```python
from build123d import *

# Parameters (mm, degrees)
SKETCH1_W           = 85
SKETCH1_H           = 45
BOSS_EXTRUDE1_DEPTH = 2
SKETCH2_W           = 52
SKETCH2_H           = 12
SKETCH2_H_2         = 4.5
SKETCH2_H_3         = 2.5
SKETCH2_H_4         = 13.8
CUT_EXTRUDE1_DEPTH  = 10
SKETCH3_W           = 85
SKETCH3_H           = 13.8
CUT_EXTRUDE2_DEPTH  = 10
SKETCH5_W           = 85
SKETCH5_H           = 5.5
CUT_EXTRUDE4_DEPTH  = 0.1
CHAMFER2_SIZE       = 0.5
CHAMFER2_SIZE2      = 2
CHAMFER3_SIZE       = 2
CHAMFER3_SIZE2      = 0.5
SKETCH8_W           = 85
SKETCH8_H           = 13.8
BOSS_EXTRUDE2_DEPTH = 2
CHAMFER4_SIZE       = 3
SKETCH6_R           = 2
CUT_EXTRUDE5_DEPTH  = 10
CUT_EXTRUDE6_DEPTH  = 6
SKETCH9_R           = 3.25
CUT_EXTRUDE8_DEPTH  = 10
SKETCH4_R           = 2.25
CUT_EXTRUDE3_DEPTH  = 10
SKETCH10_W          = 85
SKETCH10_H          = 8
CUT_EXTRUDE9_DEPTH  = 10
CHAMFER5_SIZE       = 1
CHAMFER5_SIZE2      = 5
CHAMFER6_SIZE       = 2


with BuildPart() as part:
    # Sketch1 → Boss-Extrude1 (new body)
    with BuildSketch(Plane(origin=(0, 0, 0), x_dir=(1, 0, 0), z_dir=(0, 1, 0))):
        Rectangle(SKETCH1_W, SKETCH1_H)
    extrude(amount=BOSS_EXTRUDE1_DEPTH)

    # Sketch2 → Cut-Extrude1 (cut)
    with BuildSketch(Plane(origin=(0, 2, 0), x_dir=(1, 0, 0), z_dir=(0, 1, 0))):
        with Locations((0, -16.5)):
            Rectangle(SKETCH2_W, SKETCH2_H)
        with Locations((0, -4.25)):
            Rectangle(SKETCH2_W, SKETCH2_H_2)
        with Locations((0, 1.75)):
            Rectangle(SKETCH2_W, SKETCH2_H_3)
        with Locations((0, 15.6)):
            Rectangle(SKETCH2_W, SKETCH2_H_4)
    extrude(amount=-CUT_EXTRUDE1_DEPTH, mode=Mode.SUBTRACT)

    # Sketch3 → Cut-Extrude2 (cut)
    with BuildSketch(Plane(origin=(0, 2, 0), x_dir=(1, 0, 0), z_dir=(0, 1, 0))):
        with Locations((0, 15.6)):
            Rectangle(SKETCH3_W, SKETCH3_H)
    extrude(amount=-CUT_EXTRUDE2_DEPTH, mode=Mode.SUBTRACT)

    # Sketch5 → Cut-Extrude4 (cut)
    with BuildSketch(Plane.XZ):
        with Locations((0, 0.75)):
            Rectangle(SKETCH5_W, SKETCH5_H)
    extrude(amount=-CUT_EXTRUDE4_DEPTH, mode=Mode.SUBTRACT)

    # Chamfer2
    chamfer2_edges = [part.edges().sort_by_distance(p)[0] for p in [
        (42.5, 0.05, 3.5),
    ]]
    chamfer2_side = [part.faces().sort_by_distance(p)[0] for p in [
        (42.5, 1.008447858, 6.954688763),
    ]]
    chamfer(chamfer2_edges, length=CHAMFER2_SIZE, length2=CHAMFER2_SIZE2, reference=chamfer2_side[0])

    # Chamfer3
    chamfer3_edges = [part.edges().sort_by_distance(p)[0] for p in [
        (42.5, 0.05, -2),
    ]]
    chamfer3_side = [part.faces().sort_by_distance(p)[0] for p in [
        (34.25, 0.05, -2),
    ]]
    chamfer(chamfer3_edges, length=CHAMFER3_SIZE, length2=CHAMFER3_SIZE2, reference=chamfer3_side[0])

    # Sketch8 → Boss-Extrude2 (add)
    with BuildSketch(Plane(origin=(0, 2, 0), x_dir=(1, 0, 0), z_dir=(0, 1, 0))):
        with Locations((0, 15.6)):
            Rectangle(SKETCH8_W, SKETCH8_H)
    extrude(amount=-BOSS_EXTRUDE2_DEPTH)

    # Chamfer4
    chamfer4_edges = [part.edges().sort_by_distance(p)[0] for p in [
        (-42.5, 1, -22.5),
        (42.5, 1, -22.5),
    ]]
    chamfer(chamfer4_edges, length=CHAMFER4_SIZE)

    # Sketch6 → Cut-Extrude5 (cut)
    with BuildSketch(Plane(origin=(0, 2, 0), x_dir=(1, 0, 0), z_dir=(0, 1, 0))):
        with Locations(Location((-31, 17.5, 0), (0, 0, 270))):
            Circle(SKETCH6_R)
        with Locations(Location((31, 17.5, 0), (0, 0, 270))):
            Circle(SKETCH6_R)
    extrude(amount=-CUT_EXTRUDE5_DEPTH, mode=Mode.SUBTRACT)

    # Sketch7 → Cut-Extrude6 (cut)
    with BuildSketch(Plane(origin=(0, 2, 0), x_dir=(1, 0, 0), z_dir=(0, 1, 0))):
        with BuildLine():
            Line((32, 15.5), (30, 15.5))
            ThreePointArc((30, 15.5), (28, 17.5), (30, 19.5))
            Line((30, 19.5), (32, 19.5))
            ThreePointArc((32, 19.5), (34, 17.5), (32, 15.5))
        make_face()
        with BuildLine():
            Line((-32, 15.5), (-30, 15.5))
            ThreePointArc((-30, 15.5), (-28, 17.5), (-30, 19.5))
            Line((-30, 19.5), (-32, 19.5))
            ThreePointArc((-32, 19.5), (-34, 17.5), (-32, 15.5))
        make_face()
    extrude(amount=-CUT_EXTRUDE6_DEPTH, mode=Mode.SUBTRACT)

    # Sketch9 → Cut-Extrude8 (cut)
    with BuildSketch(Plane(origin=(0, 2, 0), x_dir=(1, 0, 0), z_dir=(0, 1, 0))):
        with Locations(Location((-19, 17, 0), (0, 0, 270))):
            Circle(SKETCH9_R)
        with Locations(Location((19, 17, 0), (0, 0, 270))):
            Circle(SKETCH9_R)
    extrude(amount=-CUT_EXTRUDE8_DEPTH, mode=Mode.SUBTRACT)

    # Sketch4 → Cut-Extrude3 (cut)
    with BuildSketch(Plane(origin=(0, 2, 0), x_dir=(1, 0, 0), z_dir=(0, 1, 0))):
        with Locations(Location((-31, 10.5, 0), (0, 0, 270))):
            Circle(SKETCH4_R)
        with Locations(Location((31, 10.5, 0), (0, 0, 270))):
            Circle(SKETCH4_R)
    extrude(amount=-CUT_EXTRUDE3_DEPTH, mode=Mode.SUBTRACT)

    # Sketch10 → Cut-Extrude9 (cut)
    with BuildSketch(Plane(origin=(0, 2, 0), x_dir=(1, 0, 0), z_dir=(0, 1, 0))):
        with Locations((0, -18.5)):
            Rectangle(SKETCH10_W, SKETCH10_H)
    extrude(amount=-CUT_EXTRUDE9_DEPTH, mode=Mode.SUBTRACT)

    # Chamfer5
    chamfer5_edges = [part.edges().sort_by_distance(p)[0] for p in [
        (-34.25, 0, 14.5),
    ]]
    chamfer5_side = [part.faces().sort_by_distance(p)[0] for p in [
        (-34.25, 1, 14.5),
    ]]
    chamfer(chamfer5_edges, length=CHAMFER5_SIZE, length2=CHAMFER5_SIZE2, reference=chamfer5_side[0])

    # Chamfer6
    chamfer6_edges = [part.edges().sort_by_distance(p)[0] for p in [
        (-26, 1.5, 14.5),
        (-42.5, 1.5, 14.5),
        (26, 1.5, 14.5),
        (42.5, 1.5, 14.5),
    ]]
    chamfer(chamfer6_edges, length=CHAMFER6_SIZE)


solid = part.part
```
Geometry: final body of the model. Coordinates: model frame, mm. A direction names the side the tool comes from. Round coordinates to 2 decimals unless told otherwise and drop trailing zeros. Write each loop counter-clockwise with the first axis right and the second up, starting at its lowest first coordinate (ties: lowest second). Pieces come first, ordered by that corner, then holes.
Item 1: Mould query, pull axis X, two halves, no side actions, for faces 4 (the face through (-1, 1, -22.5)), 5 (the face through (-31, 1, -19.5)), 6 (the face through (42.5, 1, -3)), 7 (the face through (28, 1, -17.5)). Classes: +X half, -X half, draft (parallel to the pull), parting line (faces both ways), or undercut.
Item 2: Section query C-C (z = 5.5). Return loops of the section in (x, y), plus the area to 3 significant figures.
Item 3: Section query A-A (z = -10.5). Return loops of the section in (x, y).
Item 4: Section query B-B (x = 19). Return loops of the section in (y, z).
Item 5: Section query D-D (x = 6). Return loops of the section in (y, z).
Item 6: Material intervals for L1, parallel to Z at x = -4.5, y = 0.25; L2, parallel to X at y = 1.5, z = -10.5; L3, parallel to Z at x = 16.5, y = 1.4, sorted ascending.
Item 7: Pin query (flat end, axial travel): P1, Ø3.5, axis at x = -31, z = -10.5, coming from the -Y side; P2, Ø0.6, axis at x = 3, y = 1.5, coming from the +Z side; P3, Ø3, axis at x = 4.5, z = 1, coming from the -Y side; P4, Ø12, axis at x = 16.5, z = -4.5, coming from the -Y side. Return the tip coordinate at first contact, or that it passes through.
Item 8: Set-up query: faces 1 (the face through (-26, 1, 12)), 2 (the face through (-0.59, 0.16, 10.3)), 3 (the face through (26, 1, 4)). Return all of +Z, -Z, +X, -X, +Y, -Y with unobstructed straight access to the full face (end or side cutting, diameter ignored); none if empty.
Completed:
1. face 4: draft
1. face 5: undercut
1. face 6: +X half
1. face 7: undercut
2. outline: (-42.5, 0) - (-26, 0) - (-26, 2) - (-42.5, 2) - close; (26, 0) - (42.5, 0) - (42.5, 2) - (26, 2) - close
2. area: 66.0 mm2
3. outline: (-42.5, 0) - (-33.25, 0) - (-33.25, 2) - (-42.5, 2) - close; (-28.75, 0) - (28.75, 0) - (28.75, 2) - (-28.75, 2) - close; (33.25, 0) - (42.5, 0) - (42.5, 2) - (33.25, 2) - close
4. outline: (0, -22.5) - (2, -22.5) - (2, -20.25) - (0, -20.25) - close; (0, -13.75) - (2, -13.75) - (2, -3) - (0, -3) - close; (0, 6.5) - (2, 6.5) - (2, 10.5) - (0.2, 10.5) - (0, 9.5) - close; (0.1, -0.5) - (2, -0.5) - (2, 2) - (0.1, 2) - close
5. outline: (0, -22.5) - (2, -22.5) - (2, -3) - (0, -3) - close; (0, 6.5) - (2, 6.5) - (2, 10.5) - (0.2, 10.5) - (0, 9.5) - close; (0.1, -0.5) - (2, -0.5) - (2, 2) - (0.1, 2) - close
6. L1: z = -22.5 to -3, -0.5 to 2, 6.5 to 10.5
6. L2: x = -42.5 to -33.25, -28.75 to 28.75, 33.25 to 42.5
6. L3: z = -22.5 to -19.08, -14.92 to -3, -0.5 to 2, 6.5 to 10.5
7. P1: passes through
7. P2: stops at z = 10.5
7. P3: stops at y = 0.1
7. P4: stops at y = 0
8. face 1: +Z, +Y, -Y
8. face 2: +Z, +X, -X, -Y
8. face 3: +Y, -Y
